Design review of the part shown in the three views and the two pictorial views. Dimensions are in mm from the part's minimum x, y and z. Give positions to 0.01 mm unless a question says otherwise; leave off trailing zeros. Write each loop counter-clockwise with the first axis right and the second up, starting at its lowest first coordinate (ties: lowest second). Pieces come first, ordered by that corner, then holes.
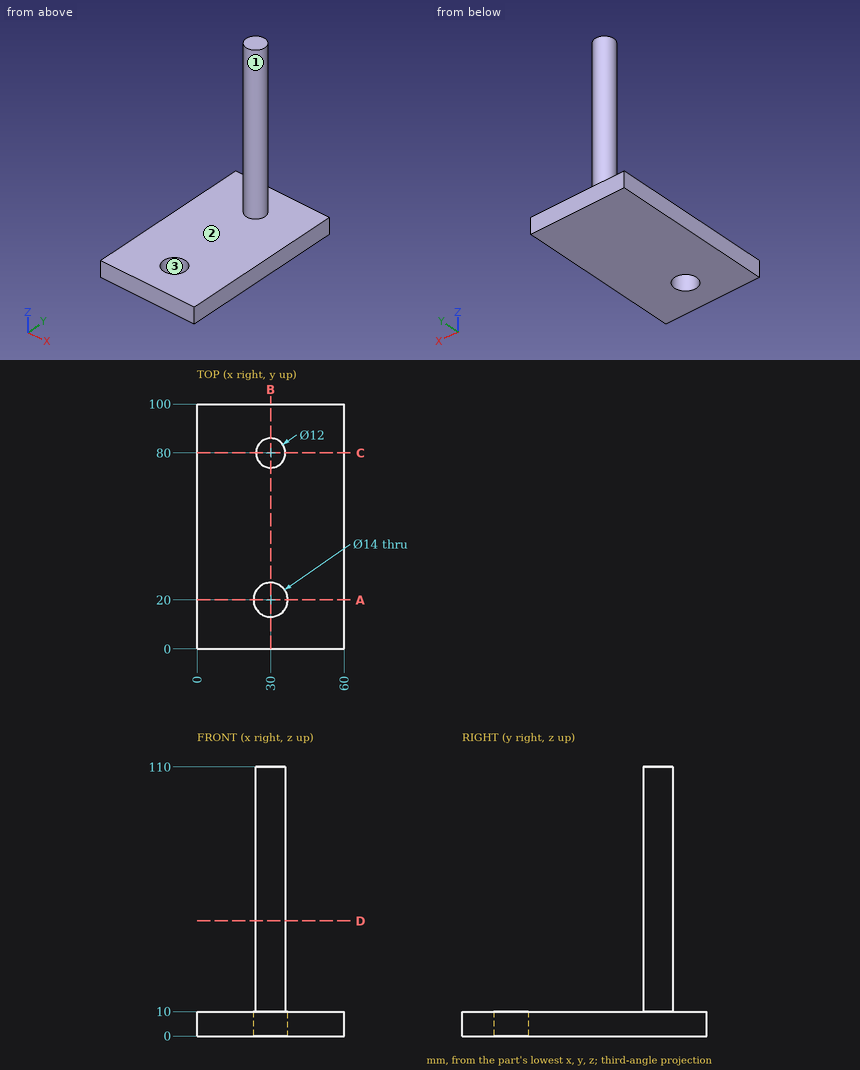
(1) Mouldability with a two-part tool opening along Y and no side actions: class the marked faces 1, 2 and 3 as pulls with the +Y half, pulls with the -Y half, needs draft (parallel to the pull), parting line crosses it, or undercut.
Resolved:
face 1: parting line crosses it
face 2: needs draft
face 3: undercut
(2) Consider section C-C, the plane y = 80. Give the boundary of the cut face in (x, z).
Resolved:
outline: (0, 0) - (60, 0) - (60, 10) - (36, 10) - (36, 110) - (24, 110) - (24, 10) - (0, 10) - close
(3) To check wall thickness, follow L1, parallel to Y at x = 30, z = 4; L2, parallel to Z at x = 4.5, y = 28; L3, parallel to Y at x = 34, z = 47. State the ranges of each line that lie inside material, in increasing order.
Resolved:
L1: y = 0 to 13, 27 to 100
L2: z = 0 to 10
L3: y = 75.53 to 84.47
(4) Consider section A-A, the plane y = 20. Give the boundary of the cut face in (x, z).
Resolved:
outline: (0, 0) - (23, 0) - (23, 10) - (0, 10) - close; (37, 0) - (60, 0) - (60, 10) - (37, 10) - close
(5) Consider section D-D, the plane z = 47. Give the boundary of the cut face in (x, y).
Resolved:
outline: circle Ø12 at (30, 80)
(6) Clearance check with flat-ended pins moving along their axes: P1, Ø1.5, axis at x = 48, y = 14.5, coming from the +Z side; P2, Ø6, axis at x = 33.5, z = 22, coming from the -Y side. State where each tip first meets the part, or that it passes through.
Resolved:
P1: stops at z = 10
P2: stops at y = 74.02
(7) Consider section B-B, the plane x = 30. Give the boundary of the cut face in (y, z), then the cut area to 3 significant figures.
Resolved:
outline: (0, 0) - (13, 0) - (13, 10) - (0, 10) - close; (27, 0) - (100, 0) - (100, 10) - (86, 10) - (86, 110) - (74, 110) - (74, 10) - (27, 10) - close
area: 2,060 mm2
